For this review, use the dimensioned drawing (mm, ordinates from the lowest corner) and the shaded views. Coordinates: 2 decimals unless noted, no trailing zeros. Write each loop counter-clockwise with the first axis right and the second up, starting at its lowest first coordinate (ties: lowest second). Pieces come first, ordered by that corner, then holes.
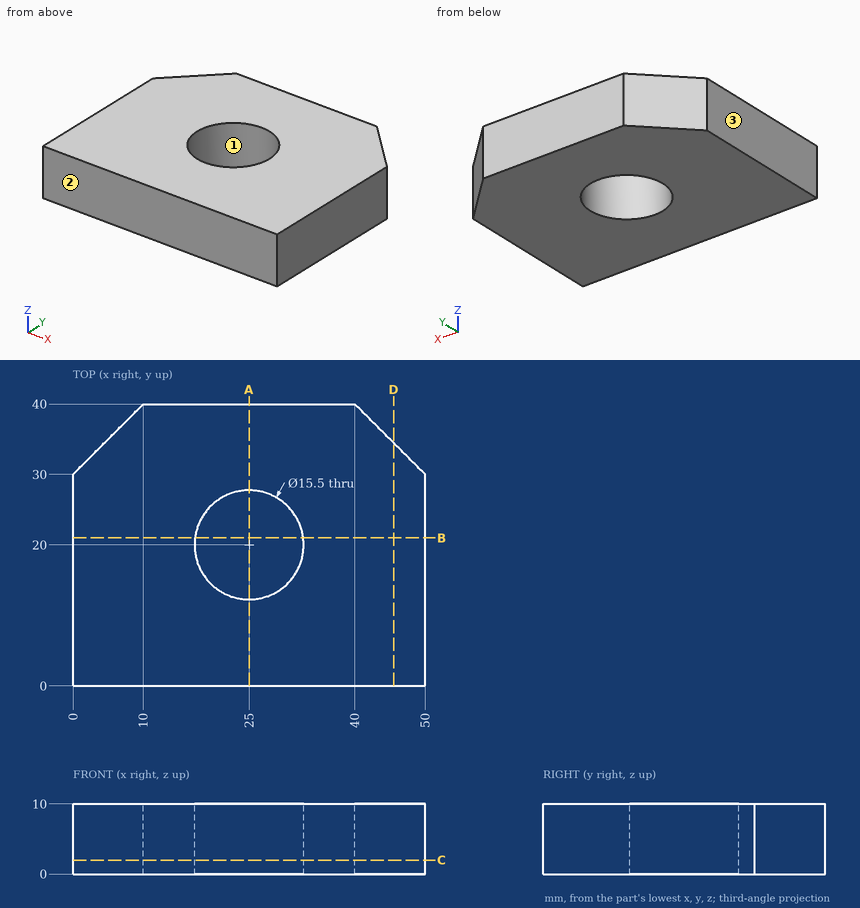
Item 1: For pin 1 (12.5 mm diameter, centred on x = 25, y = 20, fed in from -Z), flat-tipped, find the tip position at first contact; note if it passes through.
Solved:
pin 1: passes through
Item 2: To check wall thickness, follow line 1 along Y through (x, z) = (25, 2.75); line 2 along X through (y, z) = (26.5, 4); line 3 along X through (y, z) = (23, 3.75). State the ranges of each line that lie inside material, in increasing order.
Solved:
line 1: y = 0 to 12.25, 27.75 to 40
line 2: x = 0 to 20.78, 29.22 to 50
line 3: x = 0 to 17.85, 32.15 to 50
Item 3: Take a section at B-B, the plane y = 21. Write out the cut boundary in (x, z).
Solved:
outline: (0, 0) - (17.31, 0) - (17.31, 10) - (0, 10) - close; (32.69, 0) - (50, 0) - (50, 10) - (32.69, 10) - close
Item 4: Mouldability with a two-part tool opening along X and no side actions: class the marked faces 1, 2 and 3 as pulls with the +X half, pulls with the -X half, needs draft (parallel to the pull), parting line crosses it, or undercut.
Solved:
face 1: undercut
face 2: needs draft
face 3: pulls with the -X half
Item 5: Take a section at A-A, the plane x = 25. Write out the cut boundary in (y, z), plus the area to 3 significant figures.
Solved:
outline: (0, 0) - (12.25, 0) - (12.25, 10) - (0, 10) - close; (27.75, 0) - (40, 0) - (40, 10) - (27.75, 10) - close
area: 245 mm2
Item 6: Take a section at C-C, the plane z = 2. Write out the cut boundary in (x, y).
Solved:
outline: (0, 0) - (50, 0) - (50, 30) - (40, 40) - (10, 40) - (0, 30) - close; hole circle Ø15.5 at (25, 20)
Item 7: Take a section at D-D, the plane x = 45.5. Write out the cut boundary in (y, z).
Solved:
outline: (0, 0) - (34.5, 0) - (34.5, 10) - (0, 10) - close
